Model file for the job. Use its own axes, mm. A direction names the side the tool comes from. Round coordinates to 2 decimals unless told otherwise and drop trailing zeros. Order: outer loops, then holes, each group sorted by start corner. A loop starts at its lowest first (then second) coordinate and runs counter-clockwise, first axis right, second up. Notation, with made-up numbers: (-3.5, -7.5) -> (29.5, -7.5) arc R20 cw to (29.5, 28.5) -> close; hole circle Ø7 at (56.25, 33.5). An arc over 180 degrees is marked (long way). Use CSV: the item, a comma, the result in double quotes.
```python
from build123d import *

# Parameters (mm, degrees)
SKETCH1_R               = 9
BOSS_EXTRUDE1_DEPTH     = 72
CUT_EXTRUDE1_DEPTH      = 74.116345642
CUT_EXTRUDE1_DEPTH_BACK = 74.116345642
M4_TAPPED_HOLE1_REACH   = 75.116
M4_TAPPED_HOLE1_BORE_R  = 1.65
CHAMFER1_SIZE           = 2


with BuildPart() as part:
    # Sketch1 → Boss-Extrude1 (new body)
    with BuildSketch(Plane.XY):
        Circle(SKETCH1_R)
    extrude(amount=BOSS_EXTRUDE1_DEPTH)

    # Sketch2 → Cut-Extrude1 (cut, two sides: drawn at the far end of the back side and taken through both)
    with BuildSketch(Plane(origin=(0, 0, 0), x_dir=(1, 0, 0), z_dir=(0, 1, 0)).offset(-CUT_EXTRUDE1_DEPTH_BACK)):
        with BuildLine():
            ThreePointArc((-2.726987011, -58.749583333), (0, -68.05), (2.726987011, -58.749583333))
            ThreePointArc((2.726987011, -58.749583333), (0, -57), (-2.726987011, -58.749583333))
        make_face()
    extrude(amount=CUT_EXTRUDE1_DEPTH + CUT_EXTRUDE1_DEPTH_BACK, mode=Mode.SUBTRACT)

    # M4 Tapped Hole1 bore → M4 Tapped Hole1 (cut, up to next)
    with BuildSketch(Plane.XY.offset(72), mode=Mode.PRIVATE) as m4_tapped_hole1_sk1:
        Circle(M4_TAPPED_HOLE1_BORE_R)
    m4_tapped_hole1_tool1 = extrude(m4_tapped_hole1_sk1.sketch, amount=-M4_TAPPED_HOLE1_REACH, mode=Mode.PRIVATE) & part.part
    add(m4_tapped_hole1_tool1.solids().sort_by_distance((0, 0, 72))[0], mode=Mode.SUBTRACT)

    # Chamfer1
    chamfer1_edges = [part.edges().sort_by_distance(p)[0] for p in [
        (-9, 0, 0),
        (-9, 0, 72),
    ]]
    chamfer(chamfer1_edges, length=CHAMFER1_SIZE)


solid = part.part
```
Q1. Cut at A-A (x = 0). Give the cut face in (y, z), plus the area to 3 significant figures.
From the geometry:
outline,"(-9, 2) -> (-7, 0) -> (7, 0) -> (9, 2) -> (9, 57) -> (-9, 57) -> close; (-9, 68.05) -> (-1.65, 68.05) -> (-1.65, 72) -> (-7, 72) -> (-9, 70) -> close; (1.65, 68.05) -> (9, 68.05) -> (9, 70) -> (7, 72) -> (1.65, 72) -> close"
area,"1,080 mm²"
Q2. Cut at C-C (z = 63). Give the cut face in (x, y), plus the area to 3 significant figures.
From the geometry:
outline,"(-5.05, -7.45) -> (-5.05, 7.45) arc R9 ccw to start; (5.05, -7.45) arc R9 ccw to (5.05, 7.45) -> close"
area,"82.7 mm²"
Q3. Probe line 1 along Z through (x, y) = (0, 4.75); line 2 along Y through (x, z) = (0, 68.85); line 3 along Z through (x, y) = (-1.25, -1.5). List the from-to ranges inside material, lowest first.
From the geometry:
line 1,"z = 0 to 57, 68.05 to 72"
line 2,"y = -9 to -1.65, 1.65 to 9"
line 3,"z = 0 to 57.27, 67.89 to 72"
Q4. Mould opens along Z. For faces 1 (the flat face through (0, 0, 0)), 2 (the flat face through (0, 2, 72)), 3 (the cylindrical face through (-2.88, -0.13, 67.15)) say: +Z half, -Z half, draft (parallel to the pull), parting line (faces both ways), or undercut.
From the geometry:
face 1,"-Z half"
face 2,"+Z half"
face 3,"undercut"
Q5. Cut at B-B (y = 0). Give the cut face in (x, z).
From the geometry:
outline,"(-9, 2) -> (-7, 0) -> (7, 0) -> (9, 2) -> (9, 70) -> (7, 72) -> (1.65, 72) -> (1.65, 67.77) arc R5.05 cw to (2.73, 58.75) arc R3 cw to (-2.73, 58.75) arc R5.05 cw to (-1.65, 67.77) -> (-1.65, 72) -> (-7, 72) -> (-9, 70) -> close"
Q6. Which spindle directions (+Z, -Z, +X, -X, +Y, -Y) get a long thin tool onto all of the face, cutting with end or side? Do faces 4 (the cylindrical face through (4.84, 7.59, 35.52)), 5 (the cylindrical face through (1.524, -0.632, 69.913)), 6 (the cylindrical face through (0, 0, 57)). Say none if no direction does.
From the geometry:
face 4,"+Z, -Z"
face 5,"+Z"
face 6,"+Y, -Y"
Q7. Cut at D-D (z = 52.5). Give the cut face in (x, y), plus the area to 3 significant figures.
From the geometry:
outline,"circle Ø18 at (0, 0)"
area,"254 mm²"
Q8. Pin check, flat tips, straight feed: pin 1 (8 mm diameter, centred on x = 0, z = 63, fed in from -Y); pin 2 (3 mm diameter, centred on x = 3, z = 39.5, fed in from -Y); pin 3 (2 mm diameter, centred on x = 0, y = 0, fed in from +Z); pin 4 (8 mm diameter, centred on y = 5.5, z = 10, fed in from +X). Stop position of each tip, or through.
From the geometry:
pin 1,"passes through"
pin 2,"stops at y = -8.87"
pin 3,"stops at z = 57.17"
pin 4,"stops at x = 8.87"
